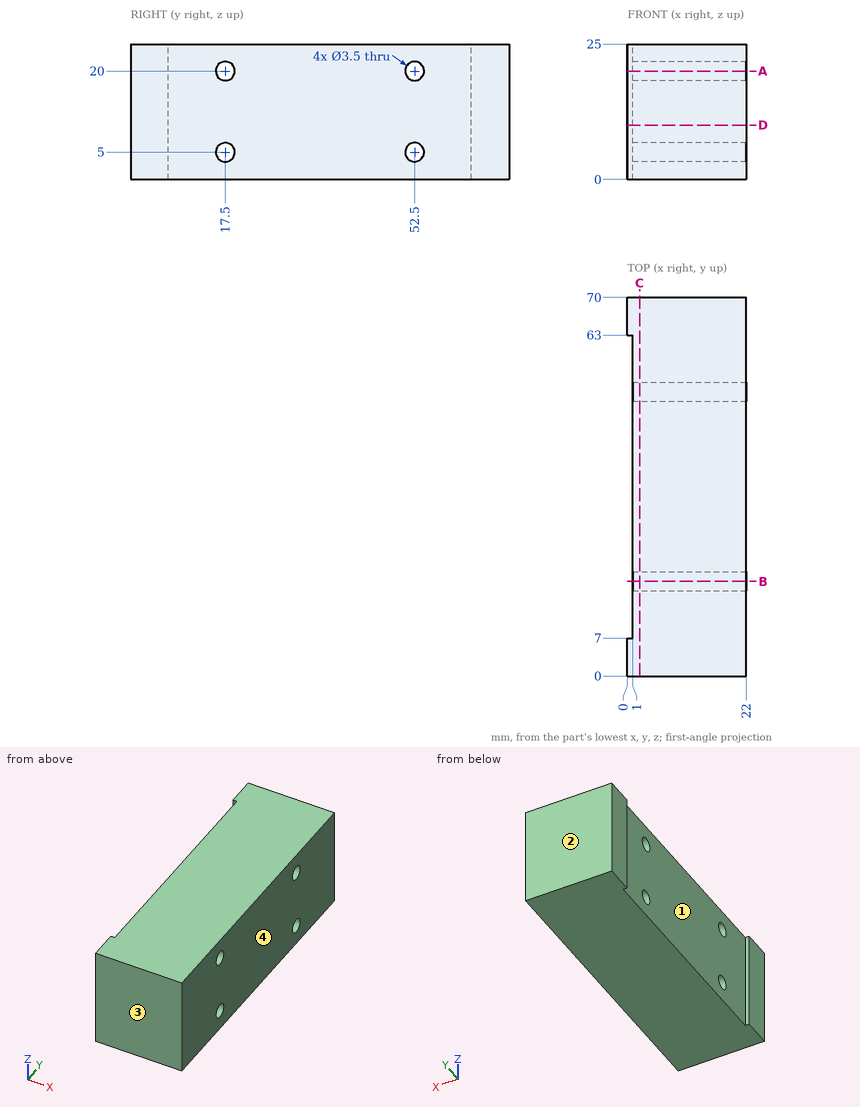
Job drawing, mm, ordinate dimensions from the low corner. One solid piece. Coordinates: 2 decimals unless noted, no trailing zeros. Write each loop counter-clockwise with the first axis right and the second up, starting at its lowest first coordinate (ties: lowest second). Pieces come first, ordered by that corner, then holes.
Item 1: Slice it at D-D (z = 10). Write the cut outline in (x, y).
Item 2: Slice it at A-A (z = 20). Write the cut outline in (x, y).
Item 3: Slice it at C-C (x = 2.25). Write the cut outline in (y, z).
Item 4: Pin check, flat tip, straight feed: pin 1 (4.5 mm diameter, centred on y = 17.5, z = 5, fed in from -X). Stop position of the tip, or through.
Item 5: Slice it at B-B (y = 17.5). Write the cut outline in (x, z).
Item 6: Probe line 1 (Y direction, x = 10, z = 5); line 2 (Z direction, x = 15.5, y = 16.5); line 3 (Z direction, x = 13.5, y = 18). List the from-to ranges inside material, lowest first.
Item 7: Mould opens along Y. For the marked faces 1, 2, 3 and 4 say: released by +Y, released by -Y, zero draft, split by the parting line, or undercut.
Results found:
1. outline: (0, 0) - (22, 0) - (22, 70) - (0, 70) - (0, 63) - (1, 63) - (1, 7) - (0, 7) - close
2. outline: (0, 0) - (22, 0) - (22, 15.75) - (1, 15.75) - (1, 7) - (0, 7) - close; (0, 63) - (1, 63) - (1, 54.25) - (22, 54.25) - (22, 70) - (0, 70) - close; (1, 19.25) - (22, 19.25) - (22, 50.75) - (1, 50.75) - close
3. outline: (0, 0) - (70, 0) - (70, 25) - (0, 25) - close; hole circle Ø3.5 at (17.5, 5); hole circle Ø3.5 at (17.5, 20); hole circle Ø3.5 at (52.5, 5); hole circle Ø3.5 at (52.5, 20)
4. pin 1: stops at x = 1
5. outline: (1, 0) - (22, 0) - (22, 3.25) - (1, 3.25) - close; (1, 6.75) - (22, 6.75) - (22, 18.25) - (1, 18.25) - close; (1, 21.75) - (22, 21.75) - (22, 25) - (1, 25) - close
6. line 1: y = 0 to 15.75, 19.25 to 50.75, 54.25 to 70
6. line 2: z = 0 to 3.56, 6.44 to 18.56, 21.44 to 25
6. line 3: z = 0 to 3.32, 6.68 to 18.32, 21.68 to 25
7. face 1: undercut
7. face 2: released by +Y
7. face 3: released by -Y
7. face 4: zero draft
